```python
from build123d import *

# Parameters (mm, degrees)
SKETCH_1_W                = 96
SKETCH_1_H                = 120
EXTRUDE_1_DEPTH           = 10
HOLE_WIZARD_2_D           = 6.4
HOLE_WIZARD_2_CBORE_D     = 11
HOLE_WIZARD_2_CBORE_DEPTH = 6.5
FILLET_1_R                = 3
HOLE_WIZARD_M4_1_D        = 3.3
SKETCH_7_R                = 2.5
CUT_EXTRUDE_1_DEPTH       = 10


with BuildPart() as part:
    # 草图1 → 凸台-拉伸1 (new body)
    with BuildSketch(Plane.XY):
        Rectangle(SKETCH_1_W, SKETCH_1_H)
    extrude(amount=EXTRUDE_1_DEPTH)

    # 打孔尺寸(%根据)内六角圆柱头螺钉的类型2 (through all)
    with Locations(Plane.XY.offset(10)):
        with Locations((-19.5, 48.95), (20.5, 48.95), (42, 48.95), (21.5, -0.05), (-20.5, -0.05), (0.5, -27.05), (-5, -53.05)):
            CounterBoreHole(HOLE_WIZARD_2_D / 2, HOLE_WIZARD_2_CBORE_D / 2, HOLE_WIZARD_2_CBORE_DEPTH)

    # 圆角1
    fillet_1_edges = [part.edges().sort_by_distance(p)[0] for p in [
        (48, -60, 5),
        (-48, -60, 5),
        (-48, 60, 5),
        (48, 60, 5),
    ]]
    fillet(fillet_1_edges, radius=FILLET_1_R)

    # M4 螺纹孔1 (through all)
    with Locations(Plane.XY.offset(10)):
        with Locations((-35, -48), (-35, 0), (35, 0), (35, -48), (-35, 38), (35, 38), (0.5, 38)):
            Hole(HOLE_WIZARD_M4_1_D / 2)

    # 草图7 → 切除-拉伸1 (cut)
    with BuildSketch(Plane.XY.offset(10)):
        with Locations((-25, 38)):
            Circle(SKETCH_7_R)
        with Locations((25, -48)):
            Circle(SKETCH_7_R)
    extrude(amount=-CUT_EXTRUDE_1_DEPTH, mode=Mode.SUBTRACT)


solid = part.part
```
Input: part model. Units: mm. Frame: model coordinates. A direction names the side the tool comes from. Coordinates: 2 decimals unless noted, no trailing zeros. Loops run counter-clockwise (first coordinate to the right, second up) from the corner with the lowest first, then second, coordinate; pieces in that order, holes last.
Q1. Section C-C, the plane x = 42. Return the cut outline in (y, z).
Results are:
outline: (-60, 0) - (45.75, 0) - (45.75, 3.5) - (43.45, 3.5) - (43.45, 10) - (-60, 10) - close; (52.15, 0) - (60, 0) - (60, 10) - (54.45, 10) - (54.45, 3.5) - (52.15, 3.5) - close
Q2. Line query: line 1 along Y through (x, z) = (35, 0.5); line 2 along Y through (x, z) = (-2, 5.5); line 3 along Y through (x, z) = (19, 2.5). Output: solid intervals per line, ascending.
Results are:
line 1: y = -60 to -49.65, -46.35 to -1.65, 1.65 to 36.35, 39.65 to 60
line 2: y = -60 to -57.66, -48.44 to -31.95, -22.15 to 60
line 3: y = -60 to -2.05, 1.95 to 46.12, 51.78 to 60
Q3. Mould query, pull axis Y, two halves, no side actions, for faces 1 (the cylindrical face through (47.1, -59.14, 5.07)), 2 (the flat face through (-1, 1, 10)), 3 (the cylindrical face through (26.746, 1.602, 6.796)). Classes: +Y half, -Y half, draft (parallel to the pull), parting line (faces both ways), or undercut.
Results are:
face 1: -Y half
face 2: draft
face 3: undercut
Q4. Contact query for a flat-ended pin moving along its axis: pin 1 (6.5 mm diameter, centred on x = 0.5, y = -27.05, fed in from +Z). Output: stop coordinate, or through.
Results are:
pin 1: stops at z = 3.5
Q5. Section A-A, the plane y = 38. Return the cut outline in (x, z), and give its area (3 significant figures).
Results are:
outline: (-48, 0) - (-36.65, 0) - (-36.65, 10) - (-48, 10) - close; (-33.35, 0) - (-27.5, 0) - (-27.5, 10) - (-33.35, 10) - close; (-22.5, 0) - (-1.15, 0) - (-1.15, 10) - (-22.5, 10) - close; (2.15, 0) - (33.35, 0) - (33.35, 10) - (2.15, 10) - close; (36.65, 0) - (48, 0) - (48, 10) - (36.65, 10) - close
area: 811 mm2
Q6. Section B-B, the plane z = 1.25. Give the number of separate pieces and of enclosed holes in the cut face, and give its area (3 significant figures).
Results are:
separate pieces: 1
enclosed holes: 16
area: 11,200 mm2
Q7. Section D-D, the plane y = -53.05. Return the cut outline in (x, z).
Results are:
outline: (-48, 0) - (-8.2, 0) - (-8.2, 3.5) - (-10.5, 3.5) - (-10.5, 10) - (-48, 10) - close; (-1.8, 0) - (48, 0) - (48, 10) - (0.5, 10) - (0.5, 3.5) - (-1.8, 3.5) - close
Q8. Set-up query: faces 4 (the cylindrical face through (47.1, 59.14, 5.07)), 5 (the cylindrical face through (-6.19, -58.42, 6.8)). Return all of +Z, -Z, +X, -X, +Y, -Y with unobstructed straight access to the full face (end or side cutting, diameter ignored); none if empty.
Results are:
face 4: +Z, -Z, +X, +Y
face 5: +Z
